```python
from build123d import *

# Parameters (mm, degrees)
SKETCH1_R           = 30
BOSS_EXTRUDE1_DEPTH = 25


with BuildPart() as part:
    # Sketch1 → Boss-Extrude1 (new body)
    with BuildSketch(Plane.XY):
        with BuildLine():
            Line((0, 0), (0, 30))
            Line((0, 30), (347.698254159, 191.313124248))
            ThreePointArc((347.698254159, 191.313124248), (416.744511221, 186.68659531), (450, 126))
            Line((450, 126), (450, 0))
            Line((450, 0), (0, 0))
        make_face()
        with Locations((378, 126)):
            Circle(SKETCH1_R, mode=Mode.SUBTRACT)
    extrude(amount=BOSS_EXTRUDE1_DEPTH)


solid = part.part
```
The listing builds one solid part. Answer for the finished solid, in the listing's coordinates (mm). Coordinates: 2 decimals unless noted, no trailing zeros. Loops run counter-clockwise (first coordinate to the right, second up) from the corner with the lowest first, then second, coordinate; pieces in that order, holes last. Notation, with made-up numbers: M -31,70 L 11,70 A19 cw 11,75 Z; hole C -13,19 d6. An arc over 180 degrees is marked long. Answer as a JSON object with one key per item and string values. Group by question number.
Item 1: Determine the mould class of faces 1 (the face through (171.42, 109.53, 12.32)), 2 (the face through (354, 108, 12)), 3 (the face through (450, 64, 12)) for opening direction X: +X half, -X half, draft (parallel to the pull), parting line (faces both ways), or undercut.
Item 2: Section C-C (x = 327) is taken. Write down the section's boundary in (y, z).
Item 3: Section B-B (z = 18.75) is taken. Write down the section's boundary in (x, y), and give its area (3 significant figures).
Item 4: Each of these flat-tipped pins is pushed along its axis until it touches: P1, Ø1.5, axis at x = 327, z = 4, coming from the +Y side; P2, Ø1.5, axis at x = 344.5, z = 8, coming from the +Y side; P3, Ø10, axis at y = 48, z = 8.5, coming from the -X side. Where does it stop, or does it pass through?
Item 5: Consider L1, parallel to Y at x = 378, z = 19.25; L2, parallel to X at y = 132, z = 19.75; L3, parallel to X at y = 146, z = 1.5. Determine where each line is inside the solid, lowest interval first.
Item 6: Section D-D (x = 179.5) is taken. Write down the section's boundary in (y, z).
Item 7: Section A-A (x = 378) is taken. Write down the section's boundary in (y, z), and give its area (3 significant figures).
Solved:
{
 "1": {"face 1": "-X half", "face 2": "undercut", "face 3": "+X half"},
 "2": {"outline": "M 0,0 L 181.71,0 L 181.71,25 L 0,25 Z"},
 "3": {"outline": "M 0,0 L 450,0 L 450,126 A72 ccw 347.7,191.31 L 0,30 Z; hole C 378,126 d60", "area": "54,700 mm2"},
 "4": {"P1": "stops at y = 182.06", "P2": "stops at y = 190.18", "P3": "stops at x = 28.02"},
 "5": {"L1": "y = 0 to 96, 156 to 198", "L2": "x = 219.85 to 348.61, 407.39 to 449.75", "L3": "x = 250.03 to 355.64, 400.36 to 447.17"},
 "6": {"outline": "M 0,0 L 113.28,0 L 113.28,25 L 0,25 Z"},
 "7": {"outline": "M 0,0 L 96,0 L 96,25 L 0,25 Z; M 156,0 L 198,0 L 198,25 L 156,25 Z", "area": "3,450 mm2"}
}
